from build123d import *

# Parameters (mm, degrees)
SKETCH1_W           = 500
SKETCH1_H           = 150
BOSS_EXTRUDE1_DEPTH = 10
SKETCH2_W           = 500
SKETCH2_H           = 100
BOSS_EXTRUDE2_DEPTH = 50


with BuildPart() as part:
    # Sketch1 → Boss-Extrude1 (new body)
    with BuildSketch(Plane.XY):
        Rectangle(SKETCH1_W, SKETCH1_H)
    extrude(amount=BOSS_EXTRUDE1_DEPTH)

    # Sketch2 → Boss-Extrude2 (add)
    with BuildSketch(Plane(origin=(0, 0, 0), x_dir=(-1, 0, 0), z_dir=(0, 0, -1))):
        Rectangle(SKETCH2_W, SKETCH2_H)
    extrude(amount=BOSS_EXTRUDE2_DEPTH)


solid = part.part
Model file for the job. Use its own axes, mm. A direction names the side the tool comes from. Coordinates: 2 decimals unless noted, no trailing zeros. Order: outer loops, then holes, each group sorted by start corner. A loop starts at its lowest first (then second) coordinate and runs counter-clockwise, first axis right, second up. Notation, with made-up numbers: (46.5, 57) -> (95.5, 57) arc R22 ccw to (95.5, 73) -> close; hole circle Ø7 at (56.5, 1). An arc over 180 degrees is marked (long way). Return JSON: item names as keys, results as strings. Group by question number.
Item 1: Flat gauge pins, fed straight in: P1, Ø7.5, axis at x = 58.5, y = 66, coming from the -Z side; P2, Ø3, axis at x = -57, z = -19.5, coming from the +Y side; P3, Ø1, axis at y = 52, z = -21.5, coming from the -X side. Where does each tip first touch, or does it go through?
Item 2: Saw through at B-B on z = -14. Write the cut outline in (x, y).
Item 3: Wall check: line 1 along Z through (x, y) = (177, 62); line 2 along Y through (x, z) = (44.5, -13). Give the ranges that are in metal, low to high. Write a range as [from, to].
Item 4: Saw through at C-C on y = -57.5. Write the cut outline in (x, z), then the cut area to 3 significant figures.
Item 5: Saw through at A-A on x = -113. Write the cut outline in (y, z).
Item 6: Tool access for faces 1 (the flat face through (-3, 63, 0)), 2 (the flat face through (-3, 75, 5)), 3 (the flat face through (3, -50, -25)): list every direction of +Z, -Z, +X, -X, +Y, -Y with a clear straight run to the whole face (end or side of a thin tool).
Values found:
{
 "1": {"P1": "stops at z = 0", "P2": "stops at y = 50", "P3": "passes through"},
 "2": {"outline": "(-250, -50) -> (250, -50) -> (250, 50) -> (-250, 50) -> close"},
 "3": {"line 1": "z = [0, 10]", "line 2": "y = [-50, 50]"},
 "4": {"outline": "(-250, 0) -> (250, 0) -> (250, 10) -> (-250, 10) -> close", "area": "5,000 mm2"},
 "5": {"outline": "(-75, 0) -> (-50, 0) -> (-50, -50) -> (50, -50) -> (50, 0) -> (75, 0) -> (75, 10) -> (-75, 10) -> close"},
 "6": {"face 1": "-Z, +X, -X, +Y", "face 2": "+Z, -Z, +X, -X, +Y", "face 3": "-Z, +X, -X, -Y"}
}
